Input: part model. Units: mm. Frame: model coordinates. Round coordinates to 2 decimals unless told otherwise and drop trailing zeros. Write each loop counter-clockwise with the first axis right and the second up, starting at its lowest first coordinate (ties: lowest second). Pieces come first, ordered by that corner, then holes. Notation, with made-up numbers: M -13.75,-1 L 1.25,-1 A6 ccw 1.25,9 Z; hole C -25.75,54 d9. An arc over 180 degrees is marked long. Answer as CSV lines item,"result". Start each with the question number.
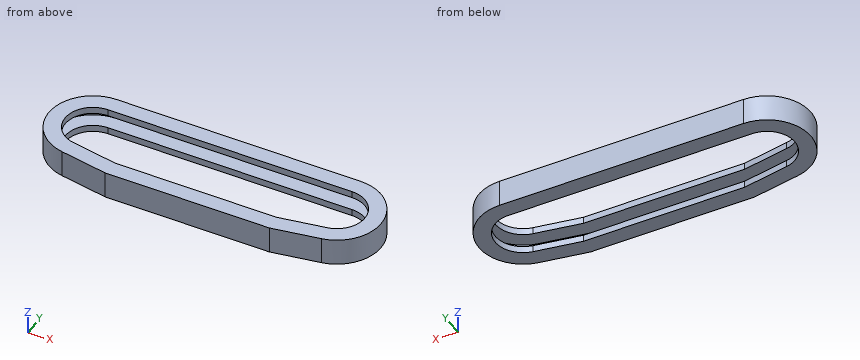
```python
from build123d import *

# Parameters (mm, degrees)
BOSS_EXTRUDE1_DEPTH = 10
CUT_EXTRUDE1_DEPTH  = 5


with BuildPart() as part:
    # Sketch2 → Boss-Extrude1 (new, symmetric)
    with BuildSketch(Plane.XY):
        with BuildLine():
            Line((-90, 32.5), (90, 32.5))
            ThreePointArc((90, 32.5), (122.376327688, 2.832561639), (95.643565774, -32.006251973))
            Line((95.643565774, -32.006251973), (60.524931981, -38.198614636))
            Line((60.524931981, -38.198614636), (-60.524931981, -38.198614636))
            Line((-60.524931981, -38.198614636), (-95.643565774, -32.006251973))
            ThreePointArc((-95.643565774, -32.006251973), (-122.376327688, 2.832561639), (-90, 32.5))
        make_face()
        with BuildLine():
            Line((-90, 20.5), (90, 20.5))
            ThreePointArc((90, 20.5), (110.421991311, 1.786692726), (93.559787642, -20.188558937))
            Line((93.559787642, -20.188558937), (59.475068019, -26.198614636))
            Line((59.475068019, -26.198614636), (-59.475068019, -26.198614636))
            Line((-59.475068019, -26.198614636), (-93.559787642, -20.188558937))
            ThreePointArc((-93.559787642, -20.188558937), (-110.421991311, 1.786692726), (-90, 20.5))
        make_face(mode=Mode.SUBTRACT)
    extrude(amount=BOSS_EXTRUDE1_DEPTH, both=True)

    # Sketch8 → Cut-Extrude1 (cut, symmetric)
    with BuildSketch(Plane.XY):
        with BuildLine():
            Line((60.437443318, -37.198614636), (95.469917597, -31.02144422))
            ThreePointArc((95.469917597, -31.02144422), (121.38013299, 2.745405897), (90, 31.5))
            Line((90, 31.5), (-90, 31.5))
            ThreePointArc((-90, 31.5), (-121.38013299, 2.745405897), (-95.469917597, -31.02144422))
            Line((-95.469917597, -31.02144422), (-60.437443318, -37.198614636))
            Line((-60.437443318, -37.198614636), (60.437443318, -37.198614636))
        make_face()
    extrude(amount=CUT_EXTRUDE1_DEPTH, both=True, mode=Mode.SUBTRACT)


solid = part.part
```
Item 1: Cut plane D-D, the plane y = 24. Return loops of the section in (x, z).
Item 2: Line query: line 1 (Y direction, x = 4, z = 2); line 2 (Z direction, x = -46, y = -29.5); line 3 (X direction, y = -1, z = 2.75). Output: solid intervals per line, ascending. Write a range as [from, to].
Item 3: Cut plane C-C, the plane y = -16. Return loops of the section in (x, z), plus the area to 3 significant figures.
Item 4: Cut plane B-B, the plane x = 45. Return loops of the section in (y, z).
Item 5: Pin query (flat end, axial travel): pin 1 Ø8 at (x, z) = (83, 7.5) entering from -Y; pin 2 Ø12 at (x, z) = (-97.5, -5.5) entering from -Y; pin 3 Ø5 at (y, z) = (-26.5, -5.5) entering from -X. Return the tip coordinate at first contact, or that it passes through.
Item 6: Cut plane A-A, the plane z = 7.5. Return loops of the section in (x, y), plus the area to 3 significant figures.
Results list:
1,outline,"M -111.91,-10 L 111.91,-10 L 111.91,10 L -111.91,10 Z; hole M -110.4,-5 L 110.4,-5 L 110.4,5 L -110.4,5 Z"
2,line 1,"[-38.2, -37.2], [31.5, 32.5]"
2,line 2,"[-10, -5], [5, 10]"
2,line 3,"[-122.48, -121.48], [121.48, 122.48]"
3,outline,"M -118.29,-10 L -102.82,-10 L -102.82,-5 L -117.13,-5 L -117.13,5 L -102.82,5 L -102.82,10 L -118.29,10 Z; M 102.82,-10 L 118.29,-10 L 118.29,10 L 102.82,10 L 102.82,5 L 117.13,5 L 117.13,-5 L 102.82,-5 Z"
3,area,"333 mm²"
4,outline,"M -38.2,-10 L -26.2,-10 L -26.2,-5 L -37.2,-5 L -37.2,5 L -26.2,5 L -26.2,10 L -38.2,10 Z; M 20.5,-10 L 32.5,-10 L 32.5,10 L 20.5,10 L 20.5,5 L 31.5,5 L 31.5,-5 L 20.5,-5 Z"
5,pin 1,"y = -34.94"
5,pin 2,"y = -32.74"
5,pin 3,"x = -111.91"
6,outline,"M -95.64,-32.01 L -60.52,-38.2 L 60.52,-38.2 L 95.64,-32.01 A32.5 ccw 90,32.5 L -90,32.5 A32.5 ccw Z; hole M -93.56,-20.19 L -59.48,-26.2 L 59.48,-26.2 L 93.56,-20.19 A20.5 ccw 90,20.5 L -90,20.5 A20.5 ccw Z"
6,area,"6,330 mm²"
